from build123d import *

# Parameters (mm, degrees)
SKETCH5_W                                         = 140
SKETCH5_H                                         = 40
BOSS_EXTRUDE1_DEPTH                               = 12
M10_CLEARANCE_HOLE1_D                             = 12
M10_CLEARANCE_HOLE1_DEPTH                         = 53
M10_CLEARANCE_HOLE1_TIP                           = 3.605163714
HOLE_SIZE_BASED_HEX_SOCKET_COUNTERSUN_D           = 11
HOLE_SIZE_BASED_HEX_SOCKET_COUNTERSUN_DEPTH       = 53
HOLE_SIZE_BASED_HEX_SOCKET_COUNTERSUN_CSINK_D     = 20.3
HOLE_SIZE_BASED_HEX_SOCKET_COUNTERSUN_CSINK_ANGLE = 90
HOLE_SIZE_BASED_HEX_SOCKET_COUNTERSUN_TIP         = 3.304733405
CHAMFER1_SIZE                                     = 2


with BuildPart() as part:
    # Sketch5 → Boss-Extrude1 (new body)
    with BuildSketch(Plane(origin=(0, 0, 0), x_dir=(1, 0, 0), z_dir=(0, 1, 0))):
        Rectangle(SKETCH5_W, SKETCH5_H)
    extrude(amount=BOSS_EXTRUDE1_DEPTH)

    # M10 Clearance Hole1
    with Locations(Plane(origin=(0, 12, 0), x_dir=(1, 0, 0), z_dir=(0, 1, 0))):
        with Locations((-55, 0), (55, 0)):
            Hole(M10_CLEARANCE_HOLE1_D / 2, depth=M10_CLEARANCE_HOLE1_DEPTH)
            with Locations((0, 0, -(M10_CLEARANCE_HOLE1_DEPTH + M10_CLEARANCE_HOLE1_TIP / 2))):  # 118° drill point
                Cone(0, M10_CLEARANCE_HOLE1_D / 2, M10_CLEARANCE_HOLE1_TIP, mode=Mode.SUBTRACT)

    # Hole size (%-based) hex socket countersunk screw type2
    with Locations(Plane(origin=(0, 0, 0), x_dir=(-1, 0, 0), z_dir=(0, -1, 0))):
        with Locations((-30, 0), (30, 0)):
            CounterSinkHole(HOLE_SIZE_BASED_HEX_SOCKET_COUNTERSUN_D / 2, HOLE_SIZE_BASED_HEX_SOCKET_COUNTERSUN_CSINK_D / 2, depth=HOLE_SIZE_BASED_HEX_SOCKET_COUNTERSUN_DEPTH, counter_sink_angle=HOLE_SIZE_BASED_HEX_SOCKET_COUNTERSUN_CSINK_ANGLE)
            with Locations((0, 0, -(HOLE_SIZE_BASED_HEX_SOCKET_COUNTERSUN_DEPTH + HOLE_SIZE_BASED_HEX_SOCKET_COUNTERSUN_TIP / 2))):  # 118° drill point
                Cone(0, HOLE_SIZE_BASED_HEX_SOCKET_COUNTERSUN_D / 2, HOLE_SIZE_BASED_HEX_SOCKET_COUNTERSUN_TIP, mode=Mode.SUBTRACT)

    # Chamfer1
    chamfer1_edges = [part.edges().sort_by_distance(p)[0] for p in [
        (70, 6, 20),
        (-70, 6, 20),
        (-70, 6, -20),
        (70, 6, -20),
    ]]
    chamfer(chamfer1_edges, length=CHAMFER1_SIZE)


solid = part.part
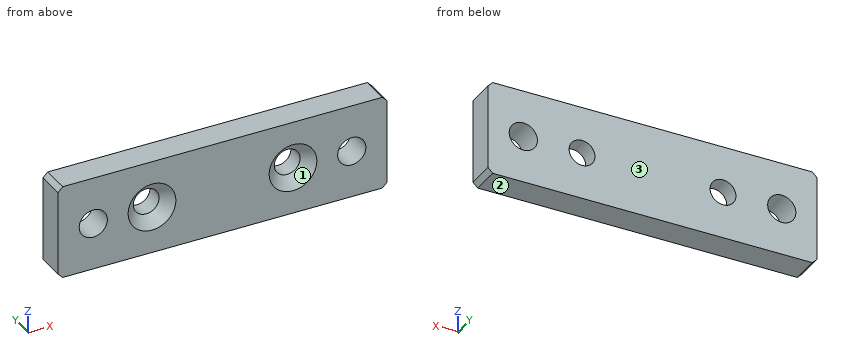
Input: part model. Units: mm. Frame: model coordinates. Face numbers are marked on the shaded views. Coordinates: 2 decimals unless noted, no trailing zeros. Loops run counter-clockwise (first coordinate to the right, second up) from the corner with the lowest first, then second, coordinate; pieces in that order, holes last.
(1) Pull-direction query (Z, two-part tool) for the marked faces 1, 2 and 3; classes: released by +Z, released by -Z, zero draft, split by the parting line, or undercut.
(2) Section C-C on z = 0. Return the cut outline in (x, y), then the cut area to 3 significant figures.
(3) Section A-A on y = 2.25. Return the cut outline in (x, z).
(4) Section D-D on x = -55. Return the cut outline in (y, z), then the cut area to 3 significant figures.
(5) Section B-B on x = -30. Return the cut outline in (y, z).
(6) Material intervals for probe 1 along Z at (x, y) = (-55, 2.5); probe 2 along Z at (x, y) = (-30, 11.25); probe 3 along X at (y, z) = (4.5, 5), sorted ascending.
(7) First-contact query: pin 1 Ø3 at (x, z) = (-16, -5.5) entering from -Y; pin 2 Ø17.5 at (x, z) = (30, 0) entering from -Y. Flat tips, straight axial feed; report the tip coordinate or a pass-through.
Data:
1. face 1: undercut
1. face 2: released by -Z
1. face 3: zero draft
2. outline: (-70, 0) - (-61, 0) - (-61, 12) - (-70, 12) - close; (-49, 0) - (-40.15, 0) - (-35.5, 4.65) - (-35.5, 12) - (-49, 12) - close; (-24.5, 4.65) - (-19.85, 0) - (19.85, 0) - (24.5, 4.65) - (24.5, 12) - (-24.5, 12) - close; (35.5, 4.65) - (40.15, 0) - (49, 0) - (49, 12) - (35.5, 12) - close; (61, 0) - (70, 0) - (70, 12) - (61, 12) - close
2. area: 1,080 mm2
3. outline: (-70, -18) - (-68, -20) - (68, -20) - (70, -18) - (70, 18) - (68, 20) - (-68, 20) - (-70, 18) - close; hole circle Ø12 at (-55, 0); hole circle Ø15.8 at (-30, 0); hole circle Ø15.8 at (30, 0); hole circle Ø12 at (55, 0)
4. outline: (0, -20) - (12, -20) - (12, -6) - (0, -6) - close; (0, 6) - (12, 6) - (12, 20) - (0, 20) - close
4. area: 336 mm2
5. outline: (0, -20) - (12, -20) - (12, -5.5) - (4.65, -5.5) - (0, -10.15) - close; (0, 10.15) - (4.65, 5.5) - (12, 5.5) - (12, 20) - (0, 20) - close
6. probe 1: z = -20 to -6, 6 to 20
6. probe 2: z = -20 to -5.5, 5.5 to 20
6. probe 3: x = -70 to -58.32, -51.68 to -32.63, -27.37 to 27.37, 32.63 to 51.68, 58.32 to 70
7. pin 1: stops at y = 0
7. pin 2: stops at y = 1.4
